```python
from build123d import *

# Parameters (mm, degrees)
SKETCH_1_W             = 35
SKETCH_1_H             = 60
EXTRUDE_1_DEPTH        = 12
CHAMFER_1_SIZE         = 2
SKETCH_4_W             = 28
SKETCH_4_H             = 12
EXTRUDE_2_DEPTH        = 35
HOLE_WIZARD_M5_1_D     = 4.2
CHAMFER_2_SIZE         = 2
HOLE_WIZARD_M5_2_D     = 4.2
HOLE_WIZARD_M5_2_DEPTH = 12.4
HOLE_WIZARD_M5_2_TIP   = 1.2618073


with BuildPart() as part:
    # 草图1 → 凸台-拉伸1 (new body)
    with BuildSketch(Plane.XY):
        Rectangle(SKETCH_1_W, SKETCH_1_H)
    extrude(amount=EXTRUDE_1_DEPTH)

    # 倒角1
    chamfer_1_edges = [part.edges().sort_by_distance(p)[0] for p in [
        (-17.5, -30, 6),
        (17.5, -30, 6),
    ]]
    chamfer(chamfer_1_edges, length=CHAMFER_1_SIZE)

    # 草图4 → 凸台-拉伸2 (add)
    with BuildSketch(Plane.ZY.offset(17.5)):
        with Locations((26, 24)):
            Rectangle(SKETCH_4_W, SKETCH_4_H)
    extrude(amount=-EXTRUDE_2_DEPTH)

    # M5 螺纹孔1 (through all)
    with Locations(Plane(origin=(0, 0, 0), x_dir=(-1, 0, 0), z_dir=(0, 0, -1))):
        with Locations((-10, -10), (10, -10)):
            Hole(HOLE_WIZARD_M5_1_D / 2)

    # 倒角2
    chamfer_2_edges = [part.edges().sort_by_distance(p)[0] for p in [
        (-17.5, 24, 40),
        (17.5, 24, 40),
    ]]
    chamfer(chamfer_2_edges, length=CHAMFER_2_SIZE)

    # M5 螺纹孔2
    with Locations(Plane(origin=(0, 30, 0), x_dir=(1, 0, 0), z_dir=(0, 1, 0))):
        with Locations((-10, -6.5), (10, -6.5), (-10, -31.5), (10, -31.5)):
            Hole(HOLE_WIZARD_M5_2_D / 2, depth=HOLE_WIZARD_M5_2_DEPTH)
            with Locations((0, 0, -(HOLE_WIZARD_M5_2_DEPTH + HOLE_WIZARD_M5_2_TIP / 2))):  # 118° drill point
                Cone(0, HOLE_WIZARD_M5_2_D / 2, HOLE_WIZARD_M5_2_TIP, mode=Mode.SUBTRACT)


solid = part.part
```
Work out the finished part from the listing and answer in its coordinate system (mm). A direction names the side the tool comes from. Give positions to 0.01 mm unless a question says otherwise; leave off trailing zeros. Loops run counter-clockwise (first coordinate to the right, second up) from the corner with the lowest first, then second, coordinate; pieces in that order, holes last. Notation, with made-up numbers: (36, -7) -> (84, -7) arc R35 cw to (84, 27) -> close; hole circle Ø11 at (77, 3). An arc over 180 degrees is marked (long way). Put each result on its own line as item: value. Start each with the question number.
Item 1: The part is cut by section B-B (z = 31.5). Give the vertices of the cut face in (x, y).
Item 2: The part is cut by section A-A (y = -10). Give the vertices of the cut face in (x, z).
Item 3: Which of the six approach directions +Z, -Z, +X, -X, +Y, -Y give full straight-line access (tool end or side, diameter ignored) to faces 1 (the face through (-8.334, 23.916, 32.778)), 2 (the face through (0, -6, 12)), 3 (the face through (12.1, 23.71, 6.41))?
Item 4: Find the intervals of material crossed by L1, parallel to Z at x = -10, y = 22; L2, parallel to Y at x = -10, z = 3.75; L3, parallel to Y at x = -13.5, z = 28.5, in increasing order. Write a range as [from, to].
Item 5: The part is cut by section C-C (x = 7). Give the vertices of the cut face in (y, z), then the cut area to 3 significant figures.
Item 6: Each of these flat-tipped pins is pushed along its axis until it touches: P1, Ø12, axis at x = -11, y = -17.5, coming from the +Z side; P2, Ø5.5, axis at x = -10, z = 31.5, coming from the +Y side; P3, Ø2, axis at x = 12.5, z = 18.5, coming from the -Y side; P4, Ø3.5, axis at x = 10, z = 31.5, coming from the -Y side. Where does it stop, or does it pass through?
Item 7: The part is cut by section D-D (z = 26). Give the vertices of the cut face in (x, y).
Item 8: The mould has two halves that part along X. Classify faces 4 (the face through (0, -30, 6)), 5 (the face through (17.5, 8, 10)), 6 (the face through (-7.9, 23.71, 6.41)): released by +X, released by -X, zero draft, split by the parting line, or undercut.
Answers below:
1. outline: (-17.5, 18) -> (-12.1, 18) -> (-12.1, 30) -> (-17.5, 30) -> close; (-7.9, 18) -> (7.9, 18) -> (7.9, 30) -> (-7.9, 30) -> close; (12.1, 18) -> (17.5, 18) -> (17.5, 30) -> (12.1, 30) -> close
2. outline: (-17.5, 0) -> (-12.1, 0) -> (-12.1, 12) -> (-17.5, 12) -> close; (-7.9, 0) -> (7.9, 0) -> (7.9, 12) -> (-7.9, 12) -> close; (12.1, 0) -> (17.5, 0) -> (17.5, 12) -> (12.1, 12) -> close
3. face 1: +Y, -Y
3. face 2: +Z, +X, -X, -Y
3. face 3: +Y
4. L1: [0, 4.4], [8.6, 29.4], [33.6, 40]
4. L2: [-30, -12.1], [-7.9, 30]
4. L3: [18, 30]
5. outline: (-30, 0) -> (30, 0) -> (30, 40) -> (18, 40) -> (18, 12) -> (-30, 12) -> close
5. area: 1,060 mm2
6. P1: z = 12
6. P2: y = 30
6. P3: y = 18
6. P4: through
7. outline: (-17.5, 18) -> (17.5, 18) -> (17.5, 30) -> (-17.5, 30) -> close
8. face 4: zero draft
8. face 5: released by +X
8. face 6: undercut
